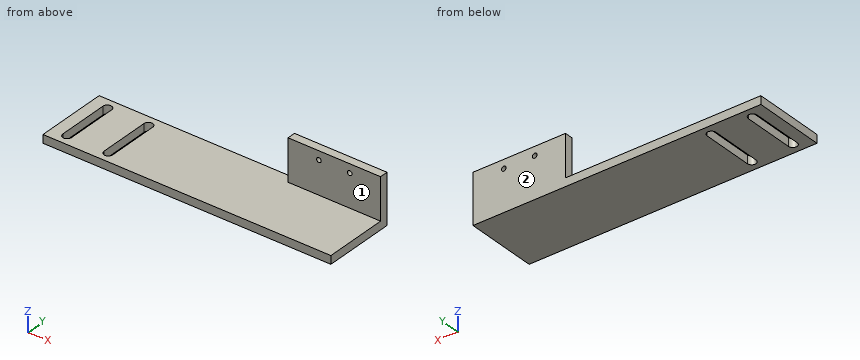
from build123d import *

# Parameters (mm, degrees)
SKETCH_1_W              = 280
SKETCH_1_H              = 70
EXTRUDE_1_DEPTH         = 8
SKETCH_2_W              = 90
SKETCH_2_H              = 8
EXTRUDE_2_DEPTH         = 40.5
HOLE_WIZARD_4_5_4_5_1_D = 4.5


with BuildPart() as part:
    # 草图1 → 凸台-拉伸1 (new body)
    with BuildSketch(Plane.XY):
        with Locations((140, 35)):
            Rectangle(SKETCH_1_W, SKETCH_1_H)
        with BuildLine():
            Line((51.5, 60), (51.5, 10))
            ThreePointArc((51.5, 10), (55.75, 5.75), (60, 10))
            Line((60, 10), (60, 60))
            ThreePointArc((60, 60), (55.75, 64.25), (51.5, 60))
        make_face(mode=Mode.SUBTRACT)
        with BuildLine():
            Line((11.5, 60), (11.5, 10))
            ThreePointArc((11.5, 10), (15.75, 5.75), (20, 10))
            Line((20, 10), (20, 60))
            ThreePointArc((20, 60), (15.75, 64.25), (11.5, 60))
        make_face(mode=Mode.SUBTRACT)
    extrude(amount=EXTRUDE_1_DEPTH)

    # 草图2 → 凸台-拉伸2 (add)
    with BuildSketch(Plane.XY.offset(8)):
        with Locations((235, 66)):
            Rectangle(SKETCH_2_W, SKETCH_2_H)
    extrude(amount=EXTRUDE_2_DEPTH)

    # Ø4.5 (4.5) 直径孔1 (through all)
    with Locations(Plane(origin=(0, 70, 0), x_dir=(-1, 0, 0), z_dir=(0, 1, 0))):
        with Locations((-220, 40), (-250, 40)):
            Hole(HOLE_WIZARD_4_5_4_5_1_D / 2)


solid = part.part
For this review, take the finished solid that the model builds, in its own axes (mm). Face numbers are marked on the shaded views. A direction names the side the tool comes from. Coordinates: 2 decimals unless noted, no trailing zeros. Loops run counter-clockwise (first coordinate to the right, second up) from the corner with the lowest first, then second, coordinate; pieces in that order, holes last. Notation, with made-up numbers: (-23.5, 31.5) - (-1.5, 31.5) arc R12 cw to (-1.5, 54.5) - close; hole circle Ø9 at (5, 16.5). An arc over 180 degrees is marked (long way). Use a Markdown table: item, result. Add a question column.
Item 1: We need section C-C (z = 11). Give the boundary of the cut face in (x, y), and give its area (3 significant figures).
Item 2: We need section A-A (y = 46). Give the boundary of the cut face in (x, z), and give its area (3 significant figures).
Item 3: Insertion check: pin 1 Ø9 at (y, z) = (64.5, 33) entering from -X; pin 2 Ø8 at (x, y) = (224.5, 39) entering from +Z; pin 3 Ø12 at (x, z) = (240.5, 25) entering from -Y. Each pin has a flat end and moves straight along its axis. Give the tip position at first contact, or say it passes through.
Item 4: We need section D-D (x = 239). Give the boundary of the cut face in (y, z), and give its area (3 significant figures).
Item 5: We need section B-B (x = 55.75). Give the boundary of the cut face in (y, z).
Item 6: For line 1 (X direction, y = 18.5, z = 6); line 2 (Z direction, x = 220, y = 67); line 3 (Z direction, x = 247, y = 50.5), list the stretches that pass through material, from the lowest coordinate up.
Item 7: Tool access review of the marked faces 1 and 2: name each direction out of +Z, -Z, +X, -X, +Y, -Y from which nothing blocks a thin tool from reaching the whole face with its end or side.
Results list:
| question | item | result |
|---|---|---|
| 1 | outline | (190, 62) - (280, 62) - (280, 70) - (190, 70) - close |
| 1 | area | 720 mm^2 |
| 2 | outline | (0, 0) - (11.5, 0) - (11.5, 8) - (0, 8) - close; (20, 0) - (51.5, 0) - (51.5, 8) - (20, 8) - close; (60, 0) - (280, 0) - (280, 8) - (60, 8) - close |
| 2 | area | 2,100 mm^2 |
| 3 | pin 1 | stops at x = 190 |
| 3 | pin 2 | stops at z = 8 |
| 3 | pin 3 | stops at y = 62 |
| 4 | outline | (0, 0) - (70, 0) - (70, 48.5) - (62, 48.5) - (62, 8) - (0, 8) - close |
| 4 | area | 884 mm^2 |
| 5 | outline | (0, 0) - (5.75, 0) - (5.75, 8) - (0, 8) - close; (64.25, 0) - (70, 0) - (70, 8) - (64.25, 8) - close |
| 6 | line 1 | x = 0 to 11.5, 20 to 51.5, 60 to 280 |
| 6 | line 2 | z = 0 to 37.75, 42.25 to 48.5 |
| 6 | line 3 | z = 0 to 8 |
| 7 | face 1 | +Z, +X, -X, -Y |
| 7 | face 2 | +Z, -Z, +X, -X, +Y |
